Check sheet for the modelled part. Datum: model origin and axes. Units: mm. A direction names the side the tool comes from. Round coordinates to 2 decimals unless told otherwise and drop trailing zeros. Write each loop counter-clockwise with the first axis right and the second up, starting at its lowest first coordinate (ties: lowest second). Pieces come first, ordered by that corner, then holes.
Item 1: Cross-section at C-C on z = 12. Enter the section's corners in (x, y), plus the area to 3 significant figures.
Item 2: Material ranges on line 1 (Z direction, x = 91.5, y = 130.5); line 2 (X direction, y = 122, z = 13); line 3 (Y direction, x = 119.5, z = 12.5), recorded low to high.
Item 3: Cross-section at A-A on x = 72.5. Enter the section's corners in (y, z), plus the area to 3 significant figures.
Item 4: Tool access check on faces 1 (the flat face through (73, 72, 15)), 2 (the cylindrical face through (84.423, 126.192, 12.465)). Record the directions out of +Z, -Z, +X, -X, +Y, -Y that give a thin tool (end or side, any length) a straight path to the whole face; none if there is none.
Item 5: Go/stop test with a flat-tipped pin: pin 1 Ø8 at (x, z) = (41.5, 11.5) entering from -Y. Record where the tip stops, or that it passes through.
from build123d import *

# Parameters (mm, degrees)
SKETCH1_W           = 145
SKETCH1_H           = 145
BOSS_EXTRUDE1_DEPTH = 10
SKETCH2_R           = 55
BOSS_EXTRUDE2_DEPTH = 5


with BuildPart() as part:
    # Sketch1 → Boss-Extrude1 (new body)
    with BuildSketch(Plane.XY):
        with Locations((72.5, 72.5)):
            Rectangle(SKETCH1_W, SKETCH1_H)
    extrude(amount=BOSS_EXTRUDE1_DEPTH)

    # Sketch2 → Boss-Extrude2 (add)
    with BuildSketch(Plane.XY.offset(10)):
        with Locations(Location((72.5, 72.5, 0), (0, 0, 180))):
            Circle(SKETCH2_R)
    extrude(amount=BOSS_EXTRUDE2_DEPTH)


solid = part.part
Response values:
1. outline: circle Ø110 at (72.5, 72.5)
1. area: 9,500 mm2
2. line 1: z = 0 to 10
2. line 2: x = 48.53 to 96.47
2. line 3: y = 43.93 to 101.07
3. outline: (0, 0) - (145, 0) - (145, 10) - (127.5, 10) - (127.5, 15) - (17.5, 15) - (17.5, 10) - (0, 10) - close
3. area: 2,000 mm2
4. face 1: +Z, +X, -X, +Y, -Y
4. face 2: +Z
5. pin 1: stops at y = 0
